Input: part model. Units: mm. Frame: model coordinates. Face numbers are marked on the shaded views. Coordinates: 2 decimals unless noted, no trailing zeros. Order: outer loops, then holes, each group sorted by start corner. A loop starts at its lowest first (then second) coordinate and runs counter-clockwise, first axis right, second up. Notation, with made-up numbers: (78, 9) - (86, 9) arc R18 cw to (86, 31) - close; hole circle Ø5 at (49.25, 37). An arc over 180 degrees is marked (long way). Answer as CSV lines item,"result". Start each with the question number.
Item 1: Section A-A (z = 62.5). Output: boundary loops of the cut face in (x, y), and give its area (3 significant figures).
Item 2: First-contact query: pin 1 (9 mm diameter, centred on x = 0, y = 15, fed in from -Z); pin 2 (5 mm diameter, centred on x = 32.88, z = -32.88, fed in from -Y). Flat tips, straight axial feed; report the tip coordinate or a pass-through.
Item 3: Section B-B (x = -13.5). Output: boundary loops of the cut face in (y, z).
Item 4: Section D-D (y = 3.5). State how many separate pieces and enclosed holes the cut face has, and give its area (3 significant figures).
Item 5: Section C-C (z = 0). Output: boundary loops of the cut face in (x, y).
Item 6: Draft query along X for the marked faces 1, 2, 3 and 4. Return one class per face: +X half, -X half, draft (parallel to the pull), parting line (faces both ways), or undercut.
Item 7: Material intervals for line 1 along X through (y, z) = (14.5, -59.5); line 2 along X through (y, z) = (20.75, -33.5); line 3 along Z through (x, y) = (45.5, 16.5), sorted ascending.
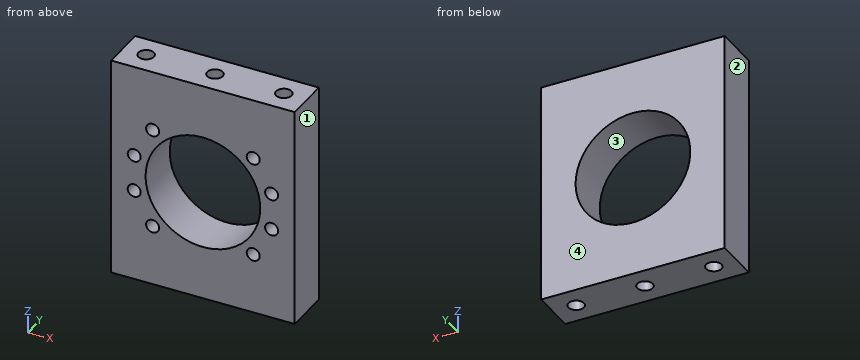
from build123d import *

# Parameters (mm, degrees)
SKETCH_1_W                   = 120
SKETCH_1_H                   = 145
SKETCH_1_R                   = 37.5
EXTRUDE_1_DEPTH              = 30
HOLE_WIZARD_M10_1_D          = 8.5
HOLE_WIZARD_M10_1_DEPTH      = 24.5
HOLE_WIZARD_M10_1_TIP        = 2.553657631
HOLE_WIZARD_M12_1_AT_2_COUNT = 2
HOLE_WIZARD_M12_1_AT_2_PITCH = 45
HOLE_WIZARD_M12_1_AT_3_COUNT = 2
HOLE_WIZARD_M12_1_AT_3_PITCH = 90


with BuildPart() as part:
    # 草图1 → 凸台-拉伸1 (new body)
    with BuildSketch(Plane(origin=(0, 0, 0), x_dir=(1, 0, 0), z_dir=(0, 1, 0))):
        Rectangle(SKETCH_1_W, SKETCH_1_H)
        with Locations(Location((0, 0, 0), (0, 0, 270))):
            Circle(SKETCH_1_R, mode=Mode.SUBTRACT)
    extrude(amount=EXTRUDE_1_DEPTH)

    # M10 螺纹孔1
    with Locations(Plane(origin=(0, 0, 0), x_dir=(-1, 0, 0), z_dir=(0, -1, 0))):
        with Locations((-32.880465325, -32.880465325), (-44.915550922, -12.035085597), (-44.915550922, 12.035085597), (-32.880465325, 32.880465325), (32.880465325, 32.880465325), (44.915550922, 12.035085597), (44.915550922, -12.035085597), (32.880465325, -32.880465325)):
            Hole(HOLE_WIZARD_M10_1_D / 2, depth=HOLE_WIZARD_M10_1_DEPTH)
            with Locations((0, 0, -(HOLE_WIZARD_M10_1_DEPTH + HOLE_WIZARD_M10_1_TIP / 2))):  # 118° drill point
                Cone(0, HOLE_WIZARD_M10_1_D / 2, HOLE_WIZARD_M10_1_TIP, mode=Mode.SUBTRACT)

    # 草图5 → M12 螺纹孔1 (revolve, cut)
    with BuildSketch(Plane(origin=(-45, 15, -72.5), x_dir=(0, 1, 0), z_dir=(1, 0, 0))):
        Polygon((0, 0), (0, 32.314389157), (5.1, 29.25), (5.1, 0), align=None)
    hole_wizard_m12_1 = revolve(axis=Axis((-45, 15, -78.85), (0, 0, 1)), mode=Mode.SUBTRACT)

    # M12 螺纹孔1 at 2: M12 螺纹孔1 ×2
    with Locations(*[(i * HOLE_WIZARD_M12_1_AT_2_PITCH, 0, 0) for i in range(1, HOLE_WIZARD_M12_1_AT_2_COUNT)]):
        add(hole_wizard_m12_1, mode=Mode.SUBTRACT)

    # M12 螺纹孔1 at 3: M12 螺纹孔1 ×2
    with Locations(*[(i * HOLE_WIZARD_M12_1_AT_3_PITCH, 0, 0) for i in range(1, HOLE_WIZARD_M12_1_AT_3_COUNT)]):
        add(hole_wizard_m12_1, mode=Mode.SUBTRACT)

    # 镜向1: M12 螺纹孔1 across plane
    add(hole_wizard_m12_1.mirror(Plane.XY), mode=Mode.SUBTRACT)

    # 镜向1 copy 1 sketch → 镜向1 copy 1 (revolve, cut)
    with BuildSketch(Plane(origin=(0, 15, 72.5), x_dir=(0, 1, 0), z_dir=(1, 0, 0))):
        Polygon((0, 0), (0, -32.314389157), (5.1, -29.25), (5.1, 0), align=None)
    revolve(axis=Axis((0, 15, 78.85), (0, 0, 1)), mode=Mode.SUBTRACT)

    # 镜向1 copy 2 sketch → 镜向1 copy 2 (revolve, cut)
    with BuildSketch(Plane(origin=(45, 15, 72.5), x_dir=(0, 1, 0), z_dir=(1, 0, 0))):
        Polygon((0, 0), (0, -32.314389157), (5.1, -29.25), (5.1, 0), align=None)
    revolve(axis=Axis((45, 15, 78.85), (0, 0, 1)), mode=Mode.SUBTRACT)


solid = part.part
Determined:
1,outline,"(-60, 0) - (60, 0) - (60, 30) - (-60, 30) - close; hole circle Ø10.2 at (-45, 15); hole circle Ø10.2 at (0, 15); hole circle Ø10.2 at (45, 15)"
1,area,"3,350 mm^2"
2,pin 1,"stops at z = -42.89"
2,pin 2,"stops at y = 25.55"
3,outline,"(0, -72.5) - (30, -72.5) - (30, -34.99) - (0, -34.99) - close; (0, 34.99) - (30, 34.99) - (30, 72.5) - (0, 72.5) - close"
4,separate pieces,"1"
4,enclosed holes,"9"
4,area,"12,500 mm^2"
5,outline,"(-60, 0) - (-37.5, 0) - (-37.5, 30) - (-60, 30) - close; (37.5, 0) - (60, 0) - (60, 30) - (37.5, 30) - close"
6,face 1,"+X half"
6,face 2,"-X half"
6,face 3,"undercut"
6,face 4,"draft"
7,line 1,"x = -60 to -50.08, -39.92 to -5.08, 5.08 to 39.92, 50.08 to 60"
7,line 2,"x = -60 to -37.09, -28.68 to -16.85, 16.85 to 28.68, 37.09 to 60"
7,line 3,"z = -41.14 to -16.24, -7.83 to 7.83, 16.24 to 41.14"
